```python
from build123d import *


with BuildPart() as part:
    # Sketch1 → Revolve1 (revolve)
    with BuildSketch(Plane.XY, mode=Mode.PRIVATE) as revolve1_sk:
        with BuildLine():
            Line((0, 0), (0, 12))
            Line((0, 12), (20, 12))
            Line((20, 12), (20, 10))
            Line((20, 10), (25.99851273, 10))
            Line((25.99851273, 10), (25.99851273, 17))
            Line((25.99851273, 17), (37.99851273, 17))
            Line((37.99851273, 17), (37.99851273, 15))
            Line((37.99851273, 15), (39.99851273, 15))
            add(Edge.make_bspline(
                [(42.56851273, 7.738055311), (41.693908377, 15), (39.99851273, 15)],
                knots=[2.112819643, 2.112819643, 2.112819643, 3.141592654, 3.141592654, 3.141592654], degree=2, weights=[1, 0.870594726, 1]))
            ThreePointArc((42.56851273, 7.738055311), (42.863176718, 6.548150813), (43.43851273, 5.465705407))
            add(Edge.make_bspline(
                [(45, 0), (45, 3.238369631), (43.43851273, 5.465705407)],
                knots=[4.71238898, 4.71238898, 4.71238898, 5.524737662, 5.524737662, 5.524737662], degree=2, weights=[1, 0.918639051, 1]))
            Line((45, 0), (0, 0))
        make_face()
    revolve(revolve1_sk.sketch.rotate(Axis((0, 0, 0), (1, 0, 0)), 180), axis=Axis((0, 0, 0), (1, 0, 0)))


solid = part.part
```
For this review, take the finished solid that the model builds, in its own axes (mm). A direction names the side the tool comes from. Round coordinates to 2 decimals unless told otherwise and drop trailing zeros. Write each loop counter-clockwise with the first axis right and the second up, starting at its lowest first coordinate (ties: lowest second). Pieces come first, ordered by that corner, then holes.
1) For line 1 along X through (y, z) = (-14, 5.5); line 2 along X through (y, z) = (-2, 7.5); line 3 along Y through (x, z) = (28, -2.5), list the stretches that pass through material, from the lowest coordinate up.
Answer below:
line 1: x = 26 to 38
line 2: x = 0 to 42.57
line 3: y = -16.82 to 16.82
2) Mouldability with a two-part tool opening along X and no side actions: class faces 1 (the face through (39.01, -8.06, -12.65)), 2 (the face through (23, 10, 0)), 3 (the face through (0, 0, 0)) as +X half, -X half, draft (parallel to the pull), parting line (faces both ways), or undercut.
Answer below:
face 1: draft
face 2: undercut
face 3: -X half
3) Machinability: for faces 4 (the face through (32.083, 2.213, -16.855)), 5 (the face through (10.14, -11.446, -3.604)), 6 (the face through (25.999, 7.3, 7.3)), 7 (the face through (37.999, -6, 14)), which of the approach directions +Z, -Z, +X, -X, +Y, -Y give a long, thin tool a straight path to every point of the face, cutting with its end or side? Answer none if there is none.
Answer below:
face 4: +X, -X
face 5: -X
face 6: none
face 7: +X
4) Insertion check: pin 1 Ø12 at (y, z) = (-10.5, -1.5) entering from +X; pin 2 Ø1 at (x, y) = (19, -1) entering from +Z; pin 3 Ø8 at (x, y) = (27, 8) entering from +Z. Each pin has a flat end and moves straight along its axis. Give the tip position at first contact, or say it passes through.
Answer below:
pin 1: stops at x = 43.95
pin 2: stops at z = 11.99
pin 3: stops at z = 16.52
5) Take a section at A-A on x = 3. Give the boundary of the cut face in (y, z).
Answer below:
outline: circle Ø24 at (0, 0)
